from build123d import *

# Parameters (mm, degrees)
SKETCH1_W           = 188
SKETCH1_H           = 40
BOSS_EXTRUDE1_DEPTH = 6
SKETCH2_R           = 4
CUT_EXTRUDE1_DEPTH  = 6
CHAMFER1_SIZE       = 2


with BuildPart() as part:
    # Sketch1 → Boss-Extrude1 (new body)
    with BuildSketch(Plane.XY):
        Rectangle(SKETCH1_W, SKETCH1_H)
    extrude(amount=BOSS_EXTRUDE1_DEPTH)

    # Sketch2 → Cut-Extrude1 (cut)
    with BuildSketch(Plane.XY.offset(6)):
        with Locations((-25, -1)):
            Circle(SKETCH2_R)
        with Locations((75, -1)):
            Circle(SKETCH2_R)
    extrude(amount=-CUT_EXTRUDE1_DEPTH, mode=Mode.SUBTRACT)

    # Chamfer1
    chamfer1_edges = [part.edges().sort_by_distance(p)[0] for p in [
        (94, -20, 3),
        (-94, -20, 3),
    ]]
    chamfer(chamfer1_edges, length=CHAMFER1_SIZE)


solid = part.part
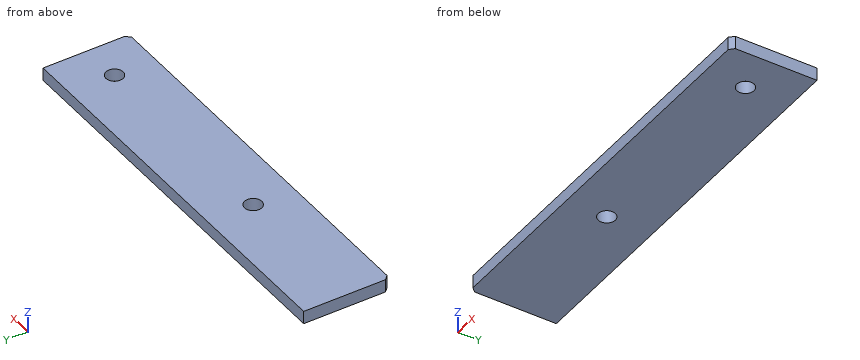
Check sheet for the modelled part. Datum: model origin and axes. Units: mm. Round coordinates to 2 decimals unless told otherwise and drop trailing zeros. Loops run counter-clockwise (first coordinate to the right, second up) from the corner with the lowest first, then second, coordinate; pieces in that order, holes last. Notation, with made-up numbers: (58, 23) -> (114, 23) arc R19 cw to (114, 51) -> close; hole circle Ø7 at (-22, -35.75). An arc over 180 degrees is marked (long way). Put each result on its own line as item: value. Start each with the question number.
1. Section check A-A (y = -1). Enter the section's corners in (x, z).
2. Scan lines: probe 1 along Y at (x, z) = (-25, 3.35); probe 2 along X at (y, z) = (1, 4.65). Record each from-to range of solid material in increasing order.
3. Gauge pin test, flat end, axial feed: pin 1 (10.5 mm diameter, centred on x = -25, y = -1, fed in from +Z). Record the tip position at first contact, or that the pin passes through.
4. Section check B-B (x = 75). Enter the section's corners in (y, z).
Findings:
1. outline: (-94, 0) -> (-29, 0) -> (-29, 6) -> (-94, 6) -> close; (-21, 0) -> (71, 0) -> (71, 6) -> (-21, 6) -> close; (79, 0) -> (94, 0) -> (94, 6) -> (79, 6) -> close
2. probe 1: y = -20 to -5, 3 to 20
2. probe 2: x = -94 to -28.46, -21.54 to 71.54, 78.46 to 94
3. pin 1: stops at z = 6
4. outline: (-20, 0) -> (-5, 0) -> (-5, 6) -> (-20, 6) -> close; (3, 0) -> (20, 0) -> (20, 6) -> (3, 6) -> close
